Verification items for this drawing (mm, ordinates from the low corner). Round coordinates to 2 decimals unless told otherwise and drop trailing zeros. Write each loop counter-clockwise with the first axis right and the second up, starting at its lowest first coordinate (ties: lowest second). Pieces come first, ordered by that corner, then holes. Notation, with made-up numbers: (14.5, 11.25) -> (44.5, 11.25) arc R31 ccw to (44.5, 47.25) -> close; hole circle Ø8 at (89, 76). An arc over 180 degrees is marked (long way). One line per item, written item: value.
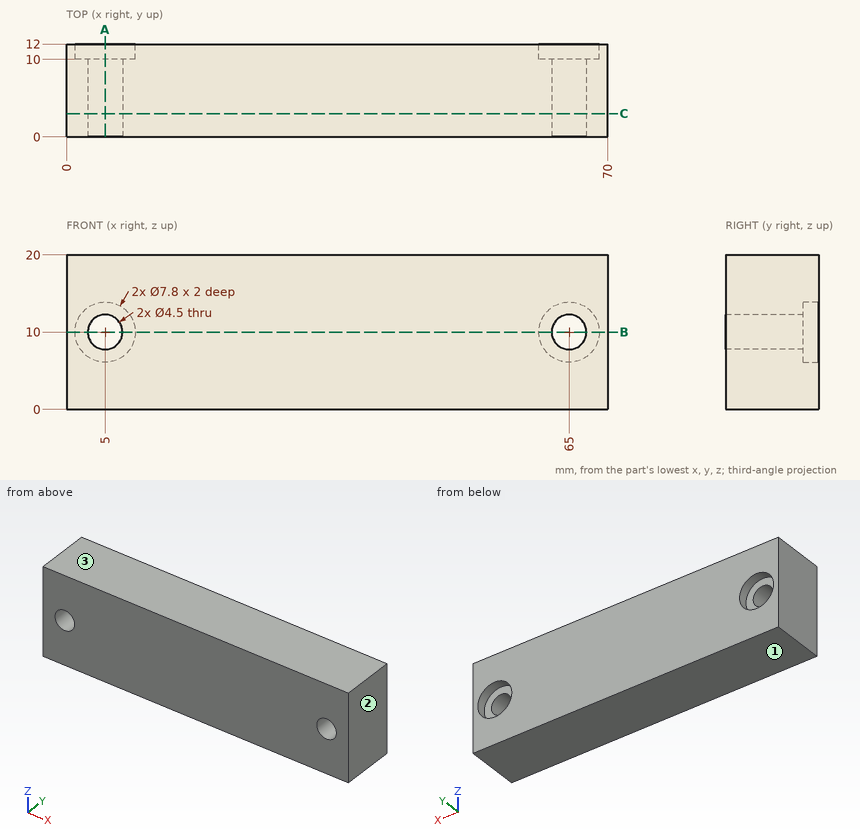
Item 1: Sectioned sample at B-B (z = 10). Enter the section's corners in (x, y).
Result set:
outline: (0, 0) -> (2.75, 0) -> (2.75, 10) -> (1.1, 10) -> (1.1, 12) -> (0, 12) -> close; (7.25, 0) -> (62.75, 0) -> (62.75, 10) -> (61.1, 10) -> (61.1, 12) -> (8.9, 12) -> (8.9, 10) -> (7.25, 10) -> close; (67.25, 0) -> (70, 0) -> (70, 12) -> (68.9, 12) -> (68.9, 10) -> (67.25, 10) -> close
Item 2: Material ranges on line 1 along X through (y, z) = (2.5, 10); line 2 along Z through (x, y) = (5, 7); line 3 along Z through (x, y) = (65, 11), recorded low to high.
Result set:
line 1: 0 to 2.75, 7.25 to 62.75, 67.25 to 70
line 2: 0 to 7.75, 12.25 to 20
line 3: 0 to 6.1, 13.9 to 20
Item 3: Sectioned sample at A-A (x = 5). Enter the section's corners in (y, z).
Result set:
outline: (0, 0) -> (12, 0) -> (12, 6.1) -> (10, 6.1) -> (10, 7.75) -> (0, 7.75) -> close; (0, 12.25) -> (10, 12.25) -> (10, 13.9) -> (12, 13.9) -> (12, 20) -> (0, 20) -> close
Item 4: Sectioned sample at C-C (y = 3). Enter the section's corners in (x, z).
Result set:
outline: (0, 0) -> (70, 0) -> (70, 20) -> (0, 20) -> close; hole circle Ø4.5 at (5, 10); hole circle Ø4.5 at (65, 10)
Item 5: Release check for a two-part mould opening along Z. For the marked faces 1, 2 and 3 record: pulls with the +Z half, pulls with the -Z half, needs draft (parallel to the pull), parting line crosses it, or undercut.
Result set:
face 1: pulls with the -Z half
face 2: needs draft
face 3: pulls with the +Z half
Item 6: Depth check by flat-ended pin: pin 1 (1.5 mm diameter, centred on x = 52, z = 17.5, fed in from -Y). Enter the tip coordinate at first touch or a pass-through.
Result set:
pin 1: y = 0
